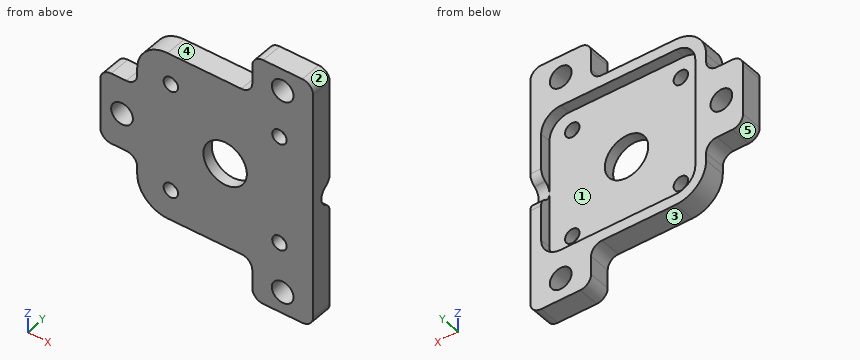
```python
from build123d import *

# Parameters (mm, degrees)
SKETCH1_W           = 81
SKETCH1_H           = 78
SKETCH1_W_2         = 71
SKETCH1_H_2         = 68
BOSS_EXTRUDE1_DEPTH = 5
SKETCH2_W           = 81
SKETCH2_H           = 78
BOSS_EXTRUDE2_DEPTH = 5
BOSS_EXTRUDE3_DEPTH = 10
FILLET1_R           = 9
FILLET2_R           = 14
FILLET4_R           = 5
SKETCH4_R           = 10
CUT_EXTRUDE1_DEPTH  = 5
SKETCH5_R           = 5
CUT_EXTRUDE2_DEPTH  = 24
SKETCH6_R           = 5
CUT_EXTRUDE3_DEPTH  = 5
FILLET5_R           = 5
SKETCH7_R           = 3.3235
CUT_EXTRUDE4_DEPTH  = 10


with BuildPart() as part:
    # Sketch1 → Boss-Extrude1 (new body)
    with BuildSketch(Plane(origin=(0, 0, 0), x_dir=(1, 0, 0), z_dir=(0, 1, 0))):
        Rectangle(SKETCH1_W, SKETCH1_H)
        Rectangle(SKETCH1_W_2, SKETCH1_H_2, mode=Mode.SUBTRACT)
    extrude(amount=BOSS_EXTRUDE1_DEPTH)

    # Sketch2 → Boss-Extrude2 (add)
    with BuildSketch(Plane.XZ):
        Rectangle(SKETCH2_W, SKETCH2_H)
    extrude(amount=BOSS_EXTRUDE2_DEPTH)

    # Sketch3 → Boss-Extrude3 (add)
    with BuildSketch(Plane.XZ.offset(5)):
        Polygon((-42.5, 16.525991305), (-57.5, 16.525991305), (-57.5, 1.525991305), (-57.5, -1.525991305), (-57.5, -16.525991305), (-43.129437713, -16.525991305), (-40.5, -16.525991305), (-40.5, 16.525991305), align=None)
        Polygon((40.5, 57.5), (12.5, 57.5), (12.5, 42.5), (12.5, 39), (40.5, 39), align=None)
        Polygon((12.5, -39), (40.5, -39), (40.5, -57.5), (12.5, -57.5), (12.5, -42.5), align=None)
    extrude(amount=-BOSS_EXTRUDE3_DEPTH)

    # Fillet1
    fillet1_edges = [part.edges().sort_by_distance(p)[0] for p in [
        (35.5, 2.5, 34),
        (35.5, 2.5, -34),
        (-35.5, 2.5, -34),
        (-35.5, 2.5, 34),
    ]]
    fillet(fillet1_edges, radius=FILLET1_R)

    # Fillet2
    fillet2_edges = [part.edges().sort_by_distance(p)[0] for p in [
        (-40.5, 0, -39),
        (-40.5, 0, 39),
    ]]
    fillet(fillet2_edges, radius=FILLET2_R)

    # Fillet4
    fillet4_edges = [part.edges().sort_by_distance(p)[0] for p in [
        (-40.5, 0, 16.525991305),
        (-40.5, 0, -16.525991305),
        (-57.5, 0, -16.525991305),
        (-57.5, 0, 16.525991305),
        (12.5, 0, -39),
        (40.5, 0, -57.5),
        (12.5, 0, -57.5),
        (12.5, 0, 57.5),
        (40.5, 0, 57.5),
        (12.5, 0, 39),
    ]]
    fillet(fillet4_edges, radius=FILLET4_R)

    # Sketch4 → Cut-Extrude1 (cut)
    with BuildSketch(Plane(origin=(0, 0, 0), x_dir=(1, 0, 0), z_dir=(0, 1, 0))):
        with Locations(Location((0, 0, 0), (0, 0, 270))):
            Circle(SKETCH4_R)
    extrude(amount=-CUT_EXTRUDE1_DEPTH, mode=Mode.SUBTRACT)

    # Sketch5 → Cut-Extrude2 (cut)
    with BuildSketch(Plane(origin=(0, 5, 0), x_dir=(1, 0, 0), z_dir=(0, 1, 0))):
        with Locations(Location((26.5, 47.5, 0), (0, 0, 270))):
            Circle(SKETCH5_R)
        with Locations(Location((26.5, -47.5, 0), (0, 0, 270))):
            Circle(SKETCH5_R)
        with Locations(Location((-47.5, 0, 0), (0, 0, 270))):
            Circle(SKETCH5_R)
    extrude(amount=-CUT_EXTRUDE2_DEPTH, mode=Mode.SUBTRACT)

    # Sketch6 → Cut-Extrude3 (cut)
    with BuildSketch(Plane(origin=(40.5, 0, 0), x_dir=(0, 0, -1), z_dir=(1, 0, 0))):
        with Locations((0, 5)):
            Circle(SKETCH6_R)
    extrude(amount=-CUT_EXTRUDE3_DEPTH, mode=Mode.SUBTRACT)

    # Fillet5
    fillet5_edges = [part.edges().sort_by_distance(p)[0] for p in [
        (38, 5, 5),
        (38, 5, -5),
    ]]
    fillet(fillet5_edges, radius=FILLET5_R)

    # Sketch7 → Cut-Extrude4 (cut)
    with BuildSketch(Plane(origin=(0, 5, 0), x_dir=(1, 0, 0), z_dir=(0, 1, 0))):
        with Locations(Location((25, 25, 0), (0, 0, 270))):
            Circle(SKETCH7_R)
        with Locations(Location((-25, 25, 0), (0, 0, 270))):
            Circle(SKETCH7_R)
        with Locations(Location((-25, -25, 0), (0, 0, 270))):
            Circle(SKETCH7_R)
        with Locations(Location((25, -25, 0), (0, 0, 270))):
            Circle(SKETCH7_R)
    extrude(amount=-CUT_EXTRUDE4_DEPTH, mode=Mode.SUBTRACT)


solid = part.part
```
Can you work these out from the model? Positions are in its coordinate system, mm. Face numbers are marked on the shaded views. A direction names the side the tool comes from. Give positions to 0.01 mm unless a question says otherwise; leave off trailing zeros. Loops run counter-clockwise (first coordinate to the right, second up) from the corner with the lowest first, then second, coordinate; pieces in that order, holes last. Notation, with made-up numbers: M 24,8.5 L 79,8.5 A23 cw 79,44.5 Z; hole C 86.5,68.25 d4. An arc over 180 degrees is marked long. One line per item, written item: value.
(1) I need wall thicknesses on line 1 (X direction, y = -2.75, z = 25); line 2 (X direction, y = -2.1, z = 0); line 3 (Z direction, x = 24.5, y = 2.25). Which ranges of each line are inside material? Lowest first, please.
Returned:
line 1: -40.5 to -28.32, -21.68 to 21.68, 28.32 to 40.5
line 2: -57.5 to -52.5, -42.5 to -10, 10 to 40.5
line 3: -57.5 to -52.08, -42.92 to -34, 34 to 42.92, 52.08 to 57.5
(2) We'd pull the mould along Z, two halves only. Please class the marked faces 1, 2 and 3: released by +Z, released by -Z, zero draft, split by the parting line, or undercut.
Returned:
face 1: undercut
face 2: released by +Z
face 3: released by -Z
(3) Suppose I cut it at B-B on y = -1.5. Count the separate pieces of the cut face and the enclosed holes in it, plus the area to 3 significant figures.
Returned:
separate pieces: 1
enclosed holes: 8
area: 7,130 mm^2
(4) Suppose I cut it at D-D on x = -47.5. List the corners of the cut face in (y, z) for me, plus the area to 3 significant figures.
Returned:
outline: M -5,-16.53 L 5,-16.53 L 5,-5 L -5,-5 Z; M -5,5 L 5,5 L 5,16.53 L -5,16.53 Z
area: 231 mm^2
(5) Which directions (+Z, -Z, +X, -X, +Y, -Y) give clear straight access to the entire face, cutting with the end or side of a thin tool? Please do the marked faces 4 and 5.
Returned:
face 4: +Z, -X, +Y, -Y
face 5: -Z, -X, +Y, -Y
(6) Suppose I cut it at A-A on z = -47.5. List the corners of the cut face in (x, y) for me, plus the area to 3 significant figures.
Returned:
outline: M 12.5,-5 L 21.5,-5 L 21.5,5 L 12.5,5 Z; M 31.5,-5 L 40.5,-5 L 40.5,5 L 31.5,5 Z
area: 180 mm^2
(7) Suppose I cut it at C-C on x = -25. List the corners of the cut face in (y, z) for me, plus the area to 3 significant figures.
Returned:
outline: M -5,-39 L 5,-39 L 5,-34 L 0,-34 L 0,-28.32 L -5,-28.32 Z; M -5,-21.68 L 0,-21.68 L 0,21.68 L -5,21.68 Z; M -5,28.32 L 0,28.32 L 0,34 L 5,34 L 5,39 L -5,39 Z
area: 374 mm^2
(8) Will these pins go through, and if not, where does the flat tip stop? pin 1 (3 mm diameter, centred on x = -5.5, y = -1, fed in from -Z); pin 2 (4 mm diameter, centred on y = 2.5, z = 16, fed in from -X) (3 decimals); pin 3 (6 mm diameter, centred on x = -25, z = 25, fed in from +Y); pin 4 (1.7 mm diameter, centred on y = 0.5, z = -23.5, fed in from -X).
Returned:
pin 1: z = -39
pin 2: x = -56.845
pin 3: through
pin 4: x = -40.5
